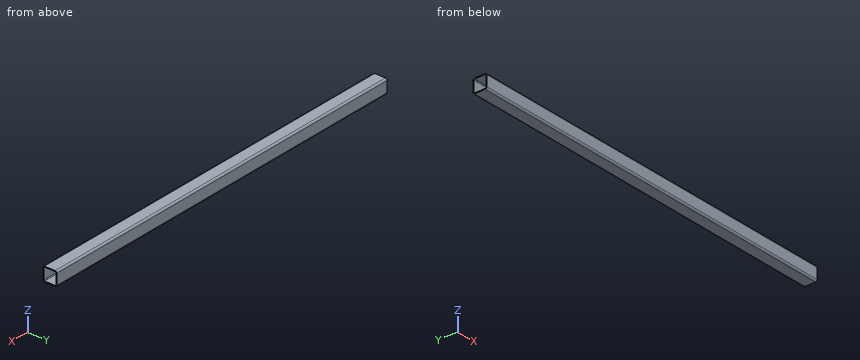
from build123d import *

# Parameters (mm, degrees)
MEMBER_30_2_1_DEPTH = 838


with BuildPart() as part:
    # Sketch1 → Member 30_2_1 (new body)
    with BuildSketch(Plane(origin=(-419, 0, 0), x_dir=(0, 0, -1), z_dir=(1, 0, 0))):
        with BuildLine():
            Line((-11.4, -15), (11.4, -15))
            ThreePointArc((11.4, -15), (13.945584412, -13.945584412), (15, -11.4))
            Line((15, -11.4), (15, 11.4))
            ThreePointArc((15, 11.4), (13.945584412, 13.945584412), (11.4, 15))
            Line((11.4, 15), (-11.4, 15))
            ThreePointArc((-11.4, 15), (-13.945584412, 13.945584412), (-15, 11.4))
            Line((-15, 11.4), (-15, -11.4))
            ThreePointArc((-15, -11.4), (-13.945584412, -13.945584412), (-11.4, -15))
        make_face()
        with BuildLine():
            Line((-11.4, -13), (11.4, -13))
            ThreePointArc((11.4, -13), (12.53137085, -12.53137085), (13, -11.4))
            Line((13, -11.4), (13, 11.4))
            ThreePointArc((13, 11.4), (12.53137085, 12.53137085), (11.4, 13))
            Line((11.4, 13), (-11.4, 13))
            ThreePointArc((-11.4, 13), (-12.53137085, 12.53137085), (-13, 11.4))
            Line((-13, 11.4), (-13, -11.4))
            ThreePointArc((-13, -11.4), (-12.53137085, -12.53137085), (-11.4, -13))
        make_face(mode=Mode.SUBTRACT)
    extrude(amount=MEMBER_30_2_1_DEPTH)


solid = part.part
Check sheet for the modelled part. Datum: model origin and axes. Units: mm. Coordinates: 2 decimals unless noted, no trailing zeros. Write each loop counter-clockwise with the first axis right and the second up, starting at its lowest first coordinate (ties: lowest second). Pieces come first, ordered by that corner, then holes.
Item 1: Scan lines: probe 1 along Y at (x, z) = (-276.5, 9); probe 2 along Z at (x, y) = (-126, -12.5). Record each from-to range of solid material in increasing order.
Numbers:
probe 1: y = -15 to -13, 13 to 15
probe 2: z = -14.83 to -12.56, 12.56 to 14.83
Item 2: Cross-section at C-C on x = 77.5. Record the boundary of the cut face in (y, z), then the cut area to 3 significant figures.
Numbers:
outline: (-15, -11.4) arc R3.6 ccw to (-11.4, -15) - (11.4, -15) arc R3.6 ccw to (15, -11.4) - (15, 11.4) arc R3.6 ccw to (11.4, 15) - (-11.4, 15) arc R3.6 ccw to (-15, 11.4) - close; hole (-13, -11.4) arc R1.6 ccw to (-11.4, -13) - (11.4, -13) arc R1.6 ccw to (13, -11.4) - (13, 11.4) arc R1.6 ccw to (11.4, 13) - (-11.4, 13) arc R1.6 ccw to (-13, 11.4) - close
area: 215 mm2
Item 3: Cross-section at A-A on z = 0. Record the boundary of the cut face in (x, y), then the cut area to 3 significant figures.
Numbers:
outline: (-419, -15) - (419, -15) - (419, -13) - (-419, -13) - close; (-419, 13) - (419, 13) - (419, 15) - (-419, 15) - close
area: 3,350 mm2
